The listing builds one solid part. Answer for the finished solid, in the listing's coordinates (mm). A direction names the side the tool comes from. Round coordinates to 2 decimals unless told otherwise and drop trailing zeros. Loops run counter-clockwise (first coordinate to the right, second up) from the corner with the lowest first, then second, coordinate; pieces in that order, holes last. Notation, with made-up numbers: (89, -27) - (106, -27) arc R26 ccw to (106, 12) - close; hole circle Ø2 at (-11.5, 51). An arc over 180 degrees is marked (long way). Write item = value, one per line. Start each with the question number.
1) Straight lines are drawn through the part: line 1 along X through (y, z) = (0.6, 0); line 2 along X through (y, z) = (1.35, -3.15); line 3 along X through (y, z) = (1.7, 0). For each, find the intervals that lie inside material, in ascending order.
2) A tool of negligible diameter and unlimited length cuts with its end or side. For faces 1 (the flat face through (4, 2, 0)), 2 (the flat face through (-8, 2.65, 0)), from which of +Z, -Z, +X, -X, +Y, -Y can it reach the whole face along a straight path? Write none if from no direction.
3) Section B-B, the plane y = 1 is taken. Determine the outline of the cut face in (x, z), and give its area (3 significant figures).
4) Given pin 1 Ø2.5 at (x, z) = (-1, 1.5) entering from +Y, flat-ended and moving along its own axis, determine where the tip first touches the part or whether it passes through.
5) For a pull along X with two mould halves and no side action, classify faces 3 (the cylindrical face through (11.66, 1.31, 0.35)), 4 (the flat face through (-12.85, 1, 0)), 5 (the flat face through (12.85, 1, 0)) as released by +X, released by -X, zero draft, split by the parting line, or undercut.
6) Section C-C, the plane x = 10.1 is taken. Determine the outline of the cut face in (y, z), and give its area (3 significant figures).
7) Section D-D, the plane z = -3.15 is taken. Determine the outline of the cut face in (x, y), and give its area (3 significant figures).
8) Section A-A, the plane z = 0 is taken. Determine the outline of the cut face in (x, y).
from build123d import *

# Parameters (mm, degrees)
SKETCH1_W           = 25.7
SKETCH1_H           = 8.3
SKETCH1_R           = 1.6
SKETCH1_R_2         = 0.6
BOSS_EXTRUDE1_DEPTH = 2.65
SKETCH2_W           = 8
SKETCH2_H           = 8.3
CUT_EXTRUDE1_DEPTH  = 1.35
CHAMFER1_SIZE       = 0.2


with BuildPart() as part:
    # Sketch1 → Boss-Extrude1 (new body)
    with BuildSketch(Plane(origin=(0, 0, 0), x_dir=(1, 0, 0), z_dir=(0, 1, 0))):
        Rectangle(SKETCH1_W, SKETCH1_H)
        with Locations(Location((-10.1, 0, 0), (0, 0, 270))):
            Circle(SKETCH1_R, mode=Mode.SUBTRACT)
        with Locations(Location((-11.35, 3.15, 0), (0, 0, 270))):
            Circle(SKETCH1_R_2, mode=Mode.SUBTRACT)
        with Locations(Location((11.35, 3.15, 0), (0, 0, 90))):
            Circle(SKETCH1_R_2, mode=Mode.SUBTRACT)
        with Locations(Location((10.1, 0, 0), (0, 0, 90))):
            Circle(SKETCH1_R, mode=Mode.SUBTRACT)
    extrude(amount=BOSS_EXTRUDE1_DEPTH)

    # Sketch2 → Cut-Extrude1 (cut)
    with BuildSketch(Plane(origin=(0, 2.65, 0), x_dir=(1, 0, 0), z_dir=(0, 1, 0))):
        Rectangle(SKETCH2_W, SKETCH2_H)
    extrude(amount=-CUT_EXTRUDE1_DEPTH, mode=Mode.SUBTRACT)

    # Chamfer1
    chamfer1_edges = [part.edges().sort_by_distance(p)[0] for p in [
        (4, 2.65, 0),
        (-4, 2.65, 0),
    ]]
    chamfer(chamfer1_edges, length=CHAMFER1_SIZE)


solid = part.part
Geometry check:
q1.line_1 = -12.85 to -11.7, -8.5 to 8.5, 11.7 to 12.85
q1.line_2 = -12.85 to -11.95, -10.75 to -4, 4 to 10.75, 11.95 to 12.85
q1.line_3 = -12.85 to -11.7, -8.5 to -4, 4 to 8.5, 11.7 to 12.85
q2.face_1 = +Z, -Z, +Y
q2.face_2 = +Z, -Z, +X, -X, +Y
q3.outline = (-12.85, -4.15) - (12.85, -4.15) - (12.85, 4.15) - (-12.85, 4.15) - close; hole circle Ø1.2 at (-11.35, -3.15); hole circle Ø3.2 at (-10.1, 0); hole circle Ø3.2 at (10.1, 0); hole circle Ø1.2 at (11.35, -3.15)
q3.area = 195 mm2
q4.pin_1 = 1.3
q5.face_3 = undercut
q5.face_4 = released by -X
q5.face_5 = released by +X
q6.outline = (0, -4.15) - (2.65, -4.15) - (2.65, -1.6) - (0, -1.6) - close; (0, 1.6) - (2.65, 1.6) - (2.65, 4.15) - (0, 4.15) - close
q6.area = 13.5 mm2
q7.outline = (-12.85, 0) - (-11.95, 0) - (-11.95, 2.65) - (-12.85, 2.65) - close; (-10.75, 0) - (10.75, 0) - (10.75, 2.65) - (4.2, 2.65) - (4, 2.45) - (4, 1.3) - (-4, 1.3) - (-4, 2.45) - (-4.2, 2.65) - (-10.75, 2.65) - close; (11.95, 0) - (12.85, 0) - (12.85, 2.65) - (11.95, 2.65) - close
q7.area = 50.9 mm2
q8.outline = (-12.85, 0) - (-11.7, 0) - (-11.7, 2.65) - (-12.85, 2.65) - close; (-8.5, 0) - (8.5, 0) - (8.5, 2.65) - (4.2, 2.65) - (4, 2.45) - (4, 1.3) - (-4, 1.3) - (-4, 2.45) - (-4.2, 2.65) - (-8.5, 2.65) - close; (11.7, 0) - (12.85, 0) - (12.85, 2.65) - (11.7, 2.65) - close
